Could you check a few things on this model? Use its own coordinates, in mm. A direction names the side the tool comes from. Round coordinates to 2 decimals unless told otherwise and drop trailing zeros. Write each loop counter-clockwise with the first axis right and the second up, starting at its lowest first coordinate (ties: lowest second). Pieces come first, ordered by that corner, then holes. Notation, with made-up numbers: (29, 34) -> (64, 34) arc R12 cw to (64, 41) -> close; hole circle Ø8 at (6.25, -19). An arc over 180 degrees is marked (long way). Return JSON: item names as keys, results as strings.
from build123d import *

# Parameters (mm, degrees)
CUT_EXTRUDE1_DEPTH = 1.5


with BuildPart() as part:
    # Sketch1 → Revolve1 (revolve)
    with BuildSketch(Plane.XY, mode=Mode.PRIVATE) as revolve1_sk:
        with BuildLine():
            Line((-2, 0), (-2, 2.75))
            Line((-2, 2.75), (0, 2.75))
            Line((0, 2.75), (0, 1.6))
            ThreePointArc((0, 1.6), (0.029289322, 1.529289322), (0.1, 1.5))
            Line((0.1, 1.5), (15.6935, 1.5))
            Line((15.6935, 1.5), (16, 1.1935))
            Line((16, 1.1935), (16, 0))
            Line((16, 0), (-2, 0))
        make_face()
    revolve(revolve1_sk.sketch.rotate(Axis((16, 0, 0), (-1, 0, 0)), 270), axis=Axis((16, 0, 0), (-1, 0, 0)))

    # Sketch2 → Cut-Revolve1 (revolve, cut)
    with BuildSketch(Plane.XY, mode=Mode.PRIVATE) as cut_revolve1_sk:
        Polygon((-2, 0), (-2, 1), (-0.5, 1), (-0.136029766, 0), align=None)
    revolve(cut_revolve1_sk.sketch.rotate(Axis((0, 0, 0), (-1, 0, 0)), 270), axis=Axis((0, 0, 0), (-1, 0, 0)), mode=Mode.SUBTRACT)

    # Sketch3 → Cut-Extrude1 (cut)
    with BuildSketch(Plane(origin=(-2, 0, 0), x_dir=(0, 0, -1), z_dir=(1, 0, 0))):
        Polygon((-1, 0.577350269), (-1, -0.577350269), (0, -1.154700538), (1, -0.577350269), (1, 0.577350269), (0, 1.154700538), align=None)
    extrude(amount=CUT_EXTRUDE1_DEPTH, mode=Mode.SUBTRACT)


solid = part.part
1) Thinking about a two-plate mould opening in Z: for faces 1 (the face through (-1.26, -0.86, 0.51)), 2 (the face through (8.01, 0.45, 1.43)), 3 (the face through (16, 0, 0)), which applies, pulls with the +Z half, pulls with the -Z half, needs draft (parallel to the pull), parting line crosses it, or undercut?
Return value:
{"face 1": "undercut", "face 2": "parting line crosses it", "face 3": "needs draft"}
2) If I drill on probe 1 along X at (y, z) = (1.3, 1.9); probe 2 along Y at (x, z) = (5.5, -1.1); probe 3 along Y at (x, z) = (-0.75, -0.1), over which ranges is the centre line in solid material (lowest first)? Write a range as [from, to].
Return value:
{"probe 1": "[-2, 0]", "probe 2": "[-1.02, 1.02]", "probe 3": "[-2.75, -1.1], [1.1, 2.75]"}
3) For faces 4 (the face through (0, 0, 2)), 5 (the face through (-2, 0, -1.2)), 6 (the face through (-1.26, 0.86, -0.51)), which set-ups out of +Z, -Z, +X, -X, +Y, -Y let a thin tool reach every point of the face, with its end or its side?
Return value:
{"face 4": "+X", "face 5": "+Z, -Z, -X, +Y, -Y", "face 6": "-X"}
4) Will these pins go through, and if not, where does the flat tip stop? pin 1 Ø2 at (y, z) = (2, 2) entering from +X; pin 2 Ø1.5 at (x, y) = (10.5, 0.5) entering from -Z; pin 3 Ø2 at (x, z) = (7, 0) entering from +Y.
Return value:
{"pin 1": "x = 0", "pin 2": "z = -1.5", "pin 3": "y = 1.5"}
5) I want a section at A-A, the plane x = 14. Please give me the cut outline in (y, z).
Return value:
{"outline": "circle Ø3 at (0, 0)"}
